from build123d import *

# Parameters (mm, degrees)
SKETCH1_R           = 7
BOSS_EXTRUDE1_DEPTH = 8


with BuildPart() as part:
    # Sketch1 → Boss-Extrude1 (new body)
    with BuildSketch(Plane.XY):
        with BuildLine():
            Line((0, 0), (-31.73420201, 0))
            ThreePointArc((-31.73420201, 0), (-39.373295872, -1.516379008), (-45.854013577, -5.835575504))
            Line((-45.854013577, -5.835575504), (-181.644244963, -141.198115671))
            Line((-181.644244963, -141.198115671), (-125.164998695, -197.855813656))
            Line((-125.164998695, -197.855813656), (-32.854013577, -105.835575504))
            ThreePointArc((-32.854013577, -105.835575504), (-26.373295872, -101.516379008), (-18.73420201, -100))
            Line((-18.73420201, -100), (0, -100))
            Line((0, -100), (0, 0))
        make_face()
        with Locations((-20, -20)):
            Circle(SKETCH1_R, mode=Mode.SUBTRACT)
        with Locations((-20, -80)):
            Circle(SKETCH1_R, mode=Mode.SUBTRACT)
    extrude(amount=BOSS_EXTRUDE1_DEPTH)


solid = part.part
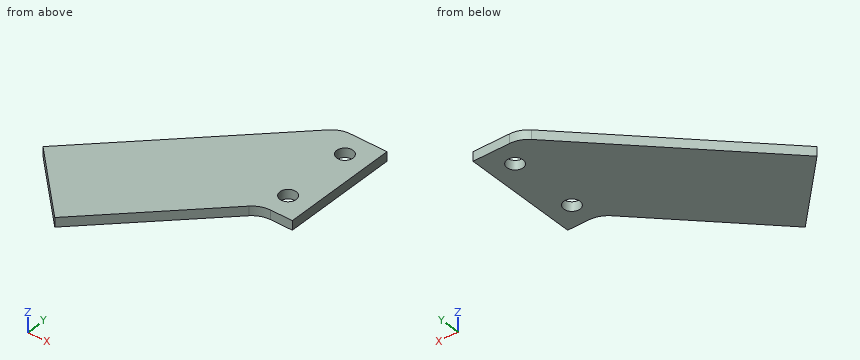
Could you check a few things on this model? Use its own coordinates, in mm. Give positions to 0.01 mm unless a question says otherwise; leave off trailing zeros. Order: outer loops, then holes, each group sorted by start corner. A loop starts at its lowest first (then second) coordinate and runs counter-clockwise, first axis right, second up.
1. Suppose I cut it at D-D (y = -76). List the corners of the cut face in (x, z) for me.
2. I need wall thicknesses on L1, parallel to Y at x = -20, z = 2.25; L2, parallel to Y at x = -12, z = 3.75; L3, parallel to X at y = -84, z = 5.75. Which ranges of each line are inside material? Lowest first, please.
3. Will these pins go through, and if not, where does the flat tip stop? P1, Ø1, axis at y = -163.5, z = 6.5, coming from the +X side; P2, Ø3, axis at y = -158, z = 6.5, coming from the -X side; P3, Ø2, axis at y = -104.5, z = 6, coming from the -X side.
4. Suppose I cut it at B-B (y = -20). List the corners of the cut face in (x, z) for me.
5. Suppose I cut it at A-A (z = 5). List the corners of the cut face in (x, y) for me (3 decimals), plus the area to 3 significant figures.
6. Suppose I cut it at C-C (x = -127.5). List the corners of the cut face in (y, z) for me, plus the area to 3 significant figures.
Solved:
1. outline: (-116.24, 0) - (-25.74, 0) - (-25.74, 8) - (-116.24, 8) - close; (-14.26, 0) - (0, 0) - (0, 8) - (-14.26, 8) - close
2. L1: y = -100.04 to -87, -73 to -27, -13 to 0
2. L2: y = -100 to 0
2. L3: x = -124.27 to -25.74, -14.26 to 0
3. P1: stops at x = -90.2
3. P2: stops at x = -166.39
3. P3: stops at x = -145.83
4. outline: (-60.06, 0) - (-27, 0) - (-27, 8) - (-60.06, 8) - close; (-13, 0) - (0, 0) - (0, 8) - (-13, 8) - close
5. outline: (-181.644, -141.198) - (-125.165, -197.856) - (-32.854, -105.836) arc R20 cw to (-18.734, -100) - (0, -100) - (0, 0) - (-31.734, 0) arc R20 ccw to (-45.854, -5.836) - close; hole circle Ø14 at (-20, -80); hole circle Ø14 at (-20, -20)
5. area: 16,600 mm2
6. outline: (-195.51, 0) - (-87.22, 0) - (-87.22, 8) - (-195.51, 8) - close
6. area: 866 mm2
